Verification items for the finished model (mm, model axes). Face numbers are marked on the shaded views. A direction names the side the tool comes from. Give positions to 0.01 mm unless a question says otherwise; leave off trailing zeros. Order: outer loops, then holes, each group sorted by start corner. A loop starts at its lowest first (then second) coordinate and runs counter-clockwise, first axis right, second up. Notation, with made-up numbers: (73.25, -26.5) - (117.25, -26.5) arc R26 cw to (117.25, 4.5) - close; hole circle Ø9 at (-19.75, 0). An arc over 180 degrees is marked (long way). Answer as a JSON object with one key per item and string values.
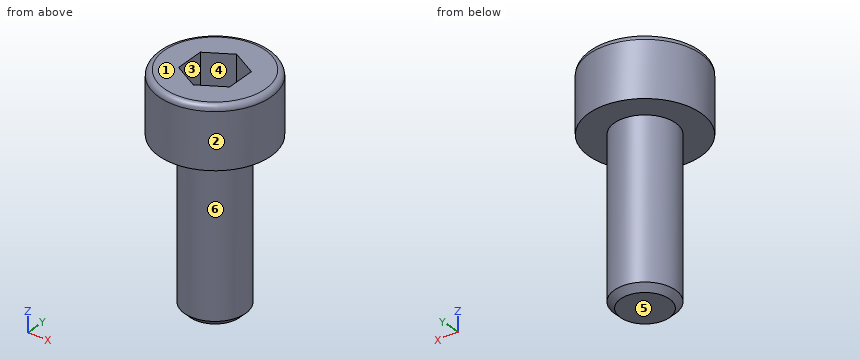
```python
from build123d import *

# Parameters (mm, degrees)
CUT_EXTRUDE_1_DEPTH = 1.925
FILLET_1_R          = 0.275
CHAMFER_1_SIZE      = 0.3


with BuildPart() as part:
    # 草图3 → 旋转1 (revolve)
    with BuildSketch(Plane(origin=(0, 0, 0), x_dir=(0, 0, -1), z_dir=(1, 0, 0)), mode=Mode.PRIVATE) as revolve_1_sk:
        Polygon((-3, 0), (-3, 2.75), (0, 2.75), (0, 1.5), (8, 1.5), (8, 0), align=None)
    revolve(revolve_1_sk.sketch.rotate(Axis((0, 0, 3), (0, 0, -1)), 180), axis=Axis((0, 0, 3), (0, 0, -1)))

    # 草图4 → 切除-拉伸1 (cut)
    with BuildSketch(Plane.XY.offset(3)):
        Polygon((0, 1.443375673), (-1.25, 0.721687836), (-1.25, -0.721687836), (0, -1.443375673), (1.25, -0.721687836), (1.25, 0.721687836), align=None)
    extrude(amount=-CUT_EXTRUDE_1_DEPTH, mode=Mode.SUBTRACT)

    # 圆角1
    fillet_1_edges = [part.edges().sort_by_distance(p)[0] for p in [
        (0, 2.75, 3),
    ]]
    fillet(fillet_1_edges, radius=FILLET_1_R)

    # 倒角1
    chamfer_1_edges = [part.edges().sort_by_distance(p)[0] for p in [
        (0, 1.5, -8),
    ]]
    chamfer(chamfer_1_edges, length=CHAMFER_1_SIZE)


solid = part.part
```
(1) Section check B-B (z = -3). Record the cut outline in (x, y).
Computed values:
{"outline": "circle Ø3 at (0, 0)"}
(2) Access from +Z, -Z, +X, -X, +Y, -Y to the whole of each face (thin tool, end or side, straight path). Record for the marked faces 4, 5 and 6.
Computed values:
{"face 4": "+Z", "face 5": "-Z, +X, -X, +Y, -Y", "face 6": "-Z"}
(3) Gauge pin test, flat ends, axial feed: pin 1 Ø1.6 at (x, y) = (1, -1) entering from -Z; pin 2 Ø1 at (x, y) = (-0.5, -2) entering from -Z; pin 3 Ø1.5 at (y, z) = (-1.5, -3) entering from -X; pin 4 Ø2 at (y, z) = (-0.5, -4.5) entering from -X. Record the tip position at first contact, or that the pin passes through.
Computed values:
{"pin 1": "stops at z = -8", "pin 2": "stops at z = 0", "pin 3": "stops at x = -1.3", "pin 4": "stops at x = -1.5"}
(4) Release check for a two-part mould opening along Y. For the marked faces 1, 2 and 3 record: pulls with the +Y half, pulls with the -Y half, needs draft (parallel to the pull), parting line crosses it, or undercut.
Computed values:
{"face 1": "needs draft", "face 2": "parting line crosses it", "face 3": "undercut"}
(5) Section check A-A (y = 0). Record the cut outline in (x, z) (3 decimals), then the cut area to 3 significant figures.
Computed values:
{"outline": "(-2.75, 0) - (-1.5, 0) - (-1.5, -7.7) - (-1.2, -8) - (1.2, -8) - (1.5, -7.7) - (1.5, 0) - (2.75, 0) - (2.75, 2.725) arc R0.275 ccw to (2.475, 3) - (1.25, 3) - (1.25, 1.075) - (-1.25, 1.075) - (-1.25, 3) - (-2.475, 3) arc R0.275 ccw to (-2.75, 2.725) - close", "area": "35.6 mm²"}
(6) Material ranges on line 1 along Z through (x, y) = (1.85, 1.2); line 2 along Z through (x, y) = (-0.4, 1.05) (3 decimals); line 3 along X through (y, z) = (0.15, 2.25), recorded low to high. Write a range as [from, to].
Computed values:
{"line 1": "z = [0, 3]", "line 2": "z = [-8, 1.075]", "line 3": "x = [-2.75, -1.25], [1.25, 2.75]"}
